Can you work these out from the model? Positions are in its coordinate system, mm. Face numbers are marked on the shaded views. A direction names the side the tool comes from. Round coordinates to 2 decimals unless told otherwise and drop trailing zeros. Loops run counter-clockwise (first coordinate to the right, second up) from the corner with the lowest first, then second, coordinate; pieces in that order, holes last. Notation, with made-up numbers: M -35.75,-39 L -3.75,-39 A18 cw -3.75,-10 Z; hole C 35,41 d4. An arc over 180 degrees is marked long. Return JSON: item names as keys, results as strings.
```python
from build123d import *

# Parameters (mm, degrees)
SKETCH1_W          = 70
SKETCH1_H          = 20
EXTRUDE1_DEPTH     = 12
CUT_EXTRUDE1_DEPTH = 39.327535793
CHAMFER1_SIZE      = 0.5


with BuildPart() as part:
    # Sketch1 → Extrude1 (new body)
    with BuildSketch(Plane(origin=(0, 0, 0), x_dir=(1, 0, 0), z_dir=(0, 1, 0))):
        Rectangle(SKETCH1_W, SKETCH1_H)
    extrude(amount=EXTRUDE1_DEPTH)

    # Sketch2 → Cut-Extrude1 (cut, through all)
    with BuildSketch(Plane(origin=(0, 12, 0), x_dir=(1, 0, 0), z_dir=(0, 1, 0))):
        with BuildLine():
            Line((22.75, 5), (22.75, -5))
            ThreePointArc((22.75, -5), (25, -7.25), (27.25, -5))
            Line((27.25, -5), (27.25, 5))
            ThreePointArc((27.25, 5), (25, 7.25), (22.75, 5))
        make_face()
        with BuildLine():
            Line((-27.25, 5), (-27.25, -5))
            ThreePointArc((-27.25, -5), (-25, -7.25), (-22.75, -5))
            Line((-22.75, -5), (-22.75, 5))
            ThreePointArc((-22.75, 5), (-25, 7.25), (-27.25, 5))
        make_face()
    extrude(amount=-CUT_EXTRUDE1_DEPTH, mode=Mode.SUBTRACT)

    # Chamfer1
    chamfer1_edges = [part.edges().sort_by_distance(p)[0] for p in [
        (35, 12, 0),
        (0, 12, -10),
        (-35, 12, 0),
        (0, 0, -10),
        (35, 0, 0),
        (0, 0, 10),
        (-35, 0, 0),
        (0, 12, 10),
        (-35, 6, -10),
        (35, 6, -10),
        (35, 6, 10),
        (-35, 6, 10),
    ]]
    chamfer(chamfer1_edges, length=CHAMFER1_SIZE)


solid = part.part
```
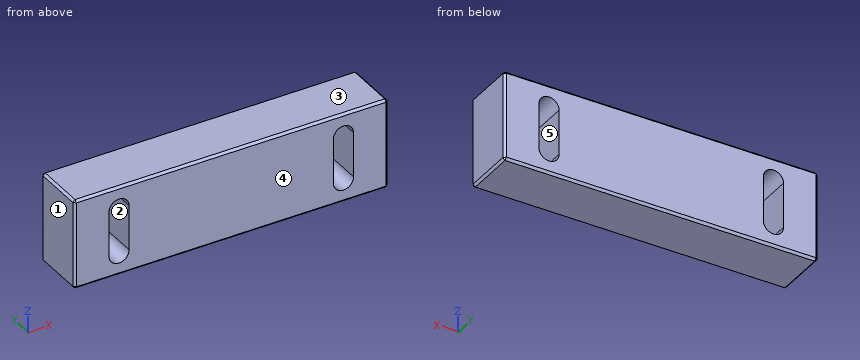
Q1. Suppose I cut it at B-B, the plane z = 0. Please give me the cut outline in (x, y), plus the area to 4 significant figures.
Results:
{"outline": "M -35,0.5 L -34.5,0 L -27.25,0 L -27.25,12 L -34.5,12 L -35,11.5 Z; M -22.75,0 L 22.75,0 L 22.75,12 L -22.75,12 Z; M 27.25,0 L 34.5,0 L 35,0.5 L 35,11.5 L 34.5,12 L 27.25,12 Z", "area": "731.5 mm2"}
Q2. Suppose I cut it at D-D, the plane x = -26. Please give me the cut outline in (y, z).
Results:
{"outline": "M 0,-9.5 L 0.5,-10 L 11.5,-10 L 12,-9.5 L 12,-7.02 L 0,-7.02 Z; M 0,7.02 L 12,7.02 L 12,9.5 L 11.5,10 L 0.5,10 L 0,9.5 Z"}
Q3. If I drill on line 1 along X through (y, z) = (9, -1.5); line 2 along X through (y, z) = (3.5, -6), over which ranges is the centre line in solid material (lowest first)?
Results:
{"line 1": "x = -35 to -27.25, -22.75 to 22.75, 27.25 to 35", "line 2": "x = -35 to -27.02, -22.98 to 22.98, 27.02 to 35"}
Q4. Suppose I cut it at C-C, the plane y = 3.5. Please give me the cut outline in (x, z).
Results:
{"outline": "M -35,-9.5 L -34.5,-10 L 34.5,-10 L 35,-9.5 L 35,9.5 L 34.5,10 L -34.5,10 L -35,9.5 Z; hole M -27.25,-5 A2.25 ccw -22.75,-5 L -22.75,5 A2.25 ccw -27.25,5 Z; hole M 22.75,-5 A2.25 ccw 27.25,-5 L 27.25,5 A2.25 ccw 22.75,5 Z"}
Q5. On a 3-axis mill with a long thin cutter (end or side, diameter ignored), from which of +Z, -Z, +X, -X, +Y, -Y can I reach the whole of each face in a straight line? I mean the marked faces 4 and 5. Say none if no direction works.
Results:
{"face 4": "+Z, -Z, +X, -X, -Y", "face 5": "+Y, -Y"}
Q6. Suppose I cut it at A-A, the plane x = 25. Please give me the cut outline in (y, z).
Results:
{"outline": "M 0,-9.5 L 0.5,-10 L 11.5,-10 L 12,-9.5 L 12,-7.25 L 0,-7.25 Z; M 0,7.25 L 12,7.25 L 12,9.5 L 11.5,10 L 0.5,10 L 0,9.5 Z"}
Q7. Thinking about a two-plate mould opening in X: for the marked faces 1, 2 and 3, which applies, pulls with the +X half, pulls with the -X half, needs draft (parallel to the pull), parting line crosses it, or undercut?
Results:
{"face 1": "pulls with the -X half", "face 2": "undercut", "face 3": "needs draft"}
